Geometry: final body of the model. Coordinates: model frame, mm. Face numbers are marked on the shaded views. A direction names the side the tool comes from. Round coordinates to 2 decimals unless told otherwise and drop trailing zeros. Write each loop counter-clockwise with the first axis right and the second up, starting at its lowest first coordinate (ties: lowest second). Pieces come first, ordered by that corner, then holes. Notation, with made-up numbers: (7, 89.25) - (58, 89.25) arc R27 ccw to (58, 126.25) - close; hole circle Ø8 at (89.25, 60). An arc over 180 degrees is marked (long way). Use a Markdown table: item, result. Add a question column.
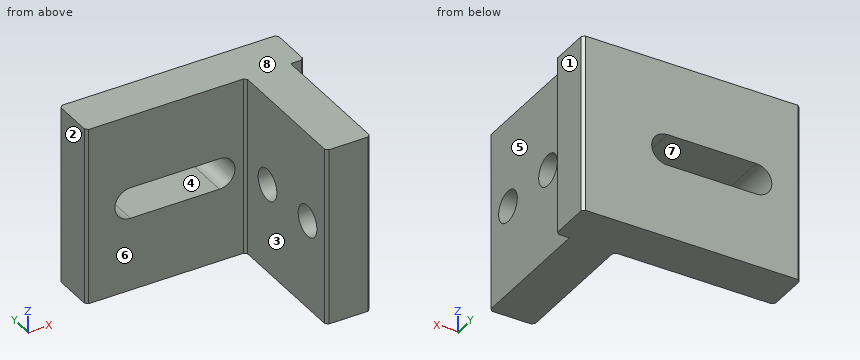
```python
from build123d import *

# Parameters (mm, degrees)
BOSS_EXTRUDE1_DEPTH = 20
CUT_EXTRUDE2_REACH  = 35.971
SKETCH2_R           = 1.75
CUT_EXTRUDE3_REACH  = 37.004


with BuildPart() as part:
    # Sketch1 → Boss-Extrude1 (new body)
    with BuildSketch(Plane.XY):
        Polygon((-6.8, 0), (-24.2, 0), (-24.5, 0.3), (-24.5, 4.7), (-24.2, 5), (-0.3, 5), (0, 4.7), (0, 0.3), (-0.3, 0), (-1.5, 0), (-1.5, -14.7), (-1.8, -15), (-6.2, -15), (-6.5, -14.7), (-6.5, -0.3), align=None)
    extrude(amount=BOSS_EXTRUDE1_DEPTH)

    # Sketch2 → Cut-Extrude2 (cut, up to next)
    with BuildSketch(Plane(origin=(-1.5, 0, 0), x_dir=(0, 0, -1), z_dir=(1, 0, 0)), mode=Mode.PRIVATE) as cut_extrude2_sk1:
        with Locations(Location((-10, -11.5, 0), (0, 0, 90))):
            Circle(SKETCH2_R)
    cut_extrude2_tool1 = extrude(cut_extrude2_sk1.sketch, amount=-CUT_EXTRUDE2_REACH, mode=Mode.PRIVATE) & part.part
    # Sketch2 → Cut-Extrude2 (cut, up to next)
    with BuildSketch(Plane(origin=(-1.5, 0, 0), x_dir=(0, 0, -1), z_dir=(1, 0, 0)), mode=Mode.PRIVATE) as cut_extrude2_sk2:
        with Locations(Location((-10, -4, 0), (0, 0, 90))):
            Circle(SKETCH2_R)
    cut_extrude2_tool2 = extrude(cut_extrude2_sk2.sketch, amount=-CUT_EXTRUDE2_REACH, mode=Mode.PRIVATE) & part.part
    add(cut_extrude2_tool1.solids().sort_by_distance((-1.5, -11.5, 10))[0], mode=Mode.SUBTRACT)
    add(cut_extrude2_tool2.solids().sort_by_distance((-1.5, -4, 10))[0], mode=Mode.SUBTRACT)

    # Sketch5 → Cut-Extrude3 (cut, up to next)
    with BuildSketch(Plane.XZ, mode=Mode.PRIVATE) as cut_extrude3_sk1:
        with BuildLine():
            Line((-19.5, 11.75), (-9.5, 11.75))
            ThreePointArc((-9.5, 11.75), (-7.75, 10), (-9.5, 8.25))
            Line((-9.5, 8.25), (-19.5, 8.25))
            ThreePointArc((-19.5, 8.25), (-21.25, 10), (-19.5, 11.75))
        make_face()
    cut_extrude3_tool1 = extrude(cut_extrude3_sk1.sketch, amount=-CUT_EXTRUDE3_REACH, mode=Mode.PRIVATE) & part.part
    add(cut_extrude3_tool1.solids().sort_by_distance((-14.5, 0, 10))[0], mode=Mode.SUBTRACT)


solid = part.part
```
1) Section A-A, the plane y = -4. Return the cut outline in (x, z), then the cut area to 3 significant figures.
2) Set-up query: the marked faces 1, 2, 3, 4 and 5. Return all of +Z, -Z, +X, -X, +Y, -Y with unobstructed straight access to the full face (end or side cutting, diameter ignored); none if empty.
3) Section C-C, the plane y = 3.5. Return the cut outline in (x, z).
4) Draft query along Z for the marked faces 6, 7 and 8. Return one class per face: released by +Z, released by -Z, zero draft, split by the parting line, or undercut.
5) Pin query (flat end, axial travel): P1, Ø5, axis at x = -15, z = 10.5, coming from the -Y side; P2, Ø3, axis at y = -11.5, z = 10, coming from the -X side; P3, Ø4.5, axis at y = -4, z = 10, coming from the -X side; P4, Ø12, axis at y = -10.5, z = 13, coming from the +X side. Return the tip coordinate at first contact, or that it passes through.
6) Section D-D, the plane x = -8.75. Return the cut outline in (y, z), then the cut area to 3 significant figures.
7) Material intervals for L1, parallel to Z at x = -4.3, y = -4; L2, parallel to X at y = -4, z = 4; L3, parallel to Y at x = -9.75, z = 1.75, sorted ascending. Write a range as from..to.
8) Section B-B, the plane z = 10. Return the cut outline in (x, y), then the cut area to 3 significant figures.
Output values:
| question | item | result |
|---|---|---|
| 1 | outline | (-6.5, 0) - (-1.5, 0) - (-1.5, 8.25) - (-6.5, 8.25) - close; (-6.5, 11.75) - (-1.5, 11.75) - (-1.5, 20) - (-6.5, 20) - close |
| 1 | area | 82.5 mm^2 |
| 2 | face 1 | +Z, -Z, +X, +Y, -Y |
| 2 | face 2 | +Z, -Z, -X, +Y, -Y |
| 2 | face 3 | +Z, -Z, -X, -Y |
| 2 | face 4 | +Y, -Y |
| 2 | face 5 | +Z, -Z, +X, -Y |
| 3 | outline | (-24.5, 0) - (0, 0) - (0, 20) - (-24.5, 20) - close; hole (-19.5, 8.25) - (-9.5, 8.25) arc R1.75 ccw to (-9.5, 11.75) - (-19.5, 11.75) arc R1.75 ccw to start |
| 4 | face 6 | zero draft |
| 4 | face 7 | undercut |
| 4 | face 8 | released by +Z |
| 5 | P1 | stops at y = 0 |
| 5 | P2 | passes through |
| 5 | P3 | stops at x = -6.5 |
| 5 | P4 | stops at x = -1.5 |
| 6 | outline | (0, 0) - (5, 0) - (5, 8.42) - (0, 8.42) - close; (0, 11.58) - (5, 11.58) - (5, 20) - (0, 20) - close |
| 6 | area | 84.2 mm^2 |
| 7 | L1 | z = 0..8.25, 11.75..20 |
| 7 | L2 | x = -6.5..-1.5 |
| 7 | L3 | y = 0..5 |
| 8 | outline | (-24.5, 0.3) - (-24.2, 0) - (-21.25, 0) - (-21.25, 5) - (-24.2, 5) - (-24.5, 4.7) - close; (-7.75, 0) - (-6.8, 0) - (-6.5, -0.3) - (-6.5, -2.25) - (-1.5, -2.25) - (-1.5, 0) - (-0.3, 0) - (0, 0.3) - (0, 4.7) - (-0.3, 5) - (-7.75, 5) - close; (-6.5, -14.7) - (-6.2, -15) - (-1.8, -15) - (-1.5, -14.7) - (-1.5, -13.25) - (-6.5, -13.25) - close; (-6.5, -9.75) - (-1.5, -9.75) - (-1.5, -5.75) - (-6.5, -5.75) - close |
| 8 | area | 94.8 mm^2 |
